from build123d import *

# Parameters (mm, degrees)
SKETCH_1_R      = 31
SKETCH_1_R_2    = 10
EXTRUDE_1_DEPTH = 25.5
SKETCH_2_R      = 5
EXTRUDE_2_DEPTH = 11
SKETCH_3_R      = 13
SKETCH_3_R_2    = 10
EXTRUDE_3_DEPTH = 7.8


with BuildPart() as part:
    # 草图1 → 凸台-拉伸1 (new body)
    with BuildSketch(Plane.XY):
        Circle(SKETCH_1_R)
        Circle(SKETCH_1_R_2, mode=Mode.SUBTRACT)
    extrude(amount=EXTRUDE_1_DEPTH)

    # 草图2 → 凸台-拉伸2 (add)
    with BuildSketch(Plane(origin=(0, 0, 0), x_dir=(-1, 0, 0), z_dir=(0, 0, -1))):
        with BuildLine():
            Line((16.881943016, 26), (52, 26))
            Line((52, 26), (74.661722806, 8.753367881))
            ThreePointArc((74.661722806, 8.753367881), (79, 0), (74.661722806, -8.753367881))
            Line((74.661722806, -8.753367881), (52, -26))
            Line((52, -26), (16.881943016, -26))
            ThreePointArc((16.881943016, -26), (31, 0), (16.881943016, 26))
        make_face()
        with Locations((69, 0)):
            Circle(SKETCH_2_R, mode=Mode.SUBTRACT)
        with Locations((42, 16)):
            Circle(SKETCH_2_R, mode=Mode.SUBTRACT)
        with Locations((42, -16)):
            Circle(SKETCH_2_R, mode=Mode.SUBTRACT)
    extrude(amount=-EXTRUDE_2_DEPTH)

    # 草图3 → 凸台-拉伸3 (add)
    with BuildSketch(Plane.XY.offset(25.5)):
        Circle(SKETCH_3_R)
        Circle(SKETCH_3_R_2, mode=Mode.SUBTRACT)
    extrude(amount=EXTRUDE_3_DEPTH)


solid = part.part
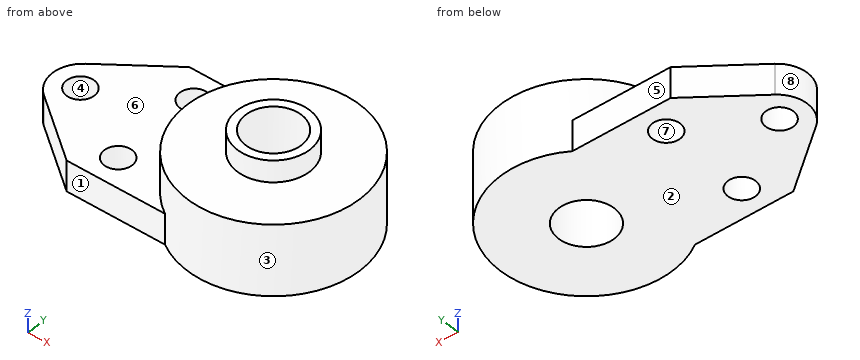
For this review, take the finished solid that the model builds, in its own axes (mm). Face numbers are marked on the shaded views. A direction names the side the tool comes from. Give positions to 0.01 mm unless a question says otherwise; leave off trailing zeros. Loops run counter-clockwise (first coordinate to the right, second up) from the corner with the lowest first, then second, coordinate; pieces in that order, holes last. Notation, with made-up numbers: M 2,63 L 21,63 A25 ccw 21,96 Z; hole C 35.25,-28.75 d8. An arc over 180 degrees is marked long. Put each result on its own line as item: value. Start each with the question number.
(1) For pin 1 (8 mm diameter, centred on x = -19, z = 23.5, fed in from -Y); pin 2 (1.5 mm diameter, centred on x = -10, z = 27.5, fed in from +Y); pin 3 (9 mm diameter, centred on x = -30, z = 7, fed in from +Y); pin 4 (13 mm diameter, centred on x = -42, y = 16, fed in from -Z), all flat-tipped, find the tip position at first contact; note any pin that passes through.
(2) Add section D-D, the plane x = 0. Write out the cut boundary in (y, z), then the cut area to 3 significant figures.
(3) Machinability: for the marked faces 1, 2, 3, 4 and 5, which of the approach directions +Z, -Z, +X, -X, +Y, -Y give a long, thin tool a straight path to every point of the face, cutting with its end or side? Answer none if there is none.
(4) Wall thickness on L1, parallel to Y at x = -42, z = 4.75; L2, parallel to Y at x = 0, z = 10; L3, parallel to Z at x = 12.5, y = 23: over which ranges is each line inside the solid? List them lowest first.
(5) Add section A-A, the plane x = -42. Write out the cut boundary in (y, z), then the cut area to 3 significant figures.
(6) Add section C-C, the plane y = 18. Write out the cut boundary in (x, z), then the cut area to 3 significant figures.
(7) The part is to be moulded in two halves that separate along Y. For the marked faces 6, 7 and 8, say which applies: +Y half, -Y half, draft (parallel to the pull), parting line (faces both ways), or undercut.
(8) Add section B-B, the plane z = 5.5. Write out the cut boundary in (x, y).
Result:
1. pin 1: stops at y = -27.13
1. pin 2: stops at y = 9.13
1. pin 3: stops at y = 26
1. pin 4: stops at z = 0
2. outline: M -31,0 L -10,0 L -10,33.3 L -13,33.3 L -13,25.5 L -31,25.5 Z; M 10,0 L 31,0 L 31,25.5 L 13,25.5 L 13,33.3 L 10,33.3 Z
2. area: 1,120 mm^2
3. face 1: +Z, -Z, -X, -Y
3. face 2: -Z, +X, -X, +Y, -Y
3. face 3: +Z
3. face 4: +Z, -Z
3. face 5: +Z, -Z, -X, +Y
4. L1: y = -26 to -21, -11 to 11, 21 to 26
4. L2: y = -31 to -10, 10 to 31
4. L3: z = 0 to 25.5
5. outline: M -26,0 L -21,0 L -21,11 L -26,11 Z; M -11,0 L 11,0 L 11,11 L -11,11 Z; M 21,0 L 26,0 L 26,11 L 21,11 Z
5. area: 352 mm^2
6. outline: M -62.51,0 L -46.58,0 L -46.58,11 L -62.51,11 Z; M -37.42,0 L 25.24,0 L 25.24,25.5 L -25.24,25.5 L -25.24,11 L -37.42,11 Z
6. area: 1,600 mm^2
7. face 6: draft
7. face 7: undercut
7. face 8: parting line
8. outline: M -74.66,-8.75 L -52,-26 L -16.88,-26 A31 ccw long -16.88,26 L -52,26 L -74.66,8.75 A11 ccw Z; hole C -69,0 d10; hole C -42,-16 d10; hole C -42,16 d10; hole C 0,0 d20
